Design review of the part built by this model. Coordinates are the model's own, in mm. A direction names the side the tool comes from. Round coordinates to 2 decimals unless told otherwise and drop trailing zeros. Loops run counter-clockwise (first coordinate to the right, second up) from the corner with the lowest first, then second, coordinate; pieces in that order, holes last. Notation, with made-up numbers: (9, -14.75) - (39, -14.75) arc R15 cw to (39, 5.25) - close; hole circle Ø8 at (28.5, -34). An arc over 180 degrees is marked (long way). Return JSON: item names as keys, results as strings. Group by question number.
(1) For faces 4 (the flat face through (10, 158, 20)), 5 (the flat face through (15, 158, 10.3)), list the 3-axis set-ups (+Z, -Z, +X, -X, +Y, -Y) from which the entire face can be reached by the end or side of a thin tool; tool diameter is ignored.
(2) We need section C-C, the plane y = 124.5. Give the number of separate pieces and of enclosed holes in the cut face, and give its area (3 significant figures).
(3) Clearance check with flat-ended pins moving along their axes: pin 1 (0.8 mm diameter, centred on y = 181, z = 17.5, fed in from +X); pin 2 (0.8 mm diameter, centred on y = 106, z = 18.5, fed in from -X); pin 3 (1.1 mm diameter, centred on y = 237.5, z = 4.5, fed in from -X). State where each tip first meets the part, or that it passes through.
(4) Wall thickness on L1, parallel to Z at x = 15, y = 106; L2, parallel to Z at x = 15.5, y = 204.5: over which ranges is each line inside the solid? List them lowest first. Write a range as [from, to].
(5) We need section A-A, the plane x = 0. Write out the cut boundary in (y, z), and give its area (3 significant figures).
(6) The part is to be moulded in two halves that separate along X. For faces 1 (the cylindrical face through (13.94, 157.76, -13.03)), 2 (the flat face through (10, 158, -20)), 3 (the flat face through (-20, 158, 10)), say which applies: pulls with the +X half, pulls with the -X half, needs draft (parallel to the pull), parting line crosses it, or undercut.
(7) We need section B-B, the plane z = 0. Write out the cut boundary in (x, y).
from build123d import *

# Parameters (mm, degrees)
SKETCH16_R     = 3.4
SKETCH16_R_2   = 3
MEMBER_1_DEPTH = 320


with BuildPart() as part:
    # Sketch16 → Member 1 (new body)
    with BuildSketch(Plane(origin=(0, 0, 0), x_dir=(-1, 0, 0), z_dir=(0, 1, 0))):
        with BuildLine():
            Line((-5.1, 20), (-5.1, 19.5))
            Line((-5.1, 19.5), (-4.1, 19.5))
            Line((-4.1, 19.5), (-4.1, 17))
            Line((-4.1, 17), (-6.1, 17))
            Line((-6.1, 17), (-6.1, 18))
            Line((-6.1, 18), (-10.3, 18))
            Line((-10.3, 18), (-10.3, 12))
            Line((-10.3, 12), (-6, 7.7))
            Line((-6, 7.7), (6, 7.7))
            Line((6, 7.7), (10.3, 12))
            Line((10.3, 12), (10.3, 18))
            Line((10.3, 18), (6.1, 18))
            Line((6.1, 18), (6.1, 17))
            Line((6.1, 17), (4.1, 17))
            Line((4.1, 17), (4.1, 19.5))
            Line((4.1, 19.5), (5.1, 19.5))
            Line((5.1, 19.5), (5.1, 20))
            Line((5.1, 20), (15.5, 20))
            ThreePointArc((15.5, 20), (18.681980515, 18.681980515), (20, 15.5))
            Line((20, 15.5), (20, 5.1))
            Line((20, 5.1), (19.5, 5.1))
            Line((19.5, 5.1), (19.5, 4.1))
            Line((19.5, 4.1), (17, 4.1))
            Line((17, 4.1), (17, 6.1))
            Line((17, 6.1), (18, 6.1))
            Line((18, 6.1), (18, 10.3))
            Line((18, 10.3), (12, 10.3))
            Line((12, 10.3), (7.7, 6))
            Line((7.7, 6), (7.7, -6))
            Line((7.7, -6), (12, -10.3))
            Line((12, -10.3), (18, -10.3))
            Line((18, -10.3), (18, -6.1))
            Line((18, -6.1), (17, -6.1))
            Line((17, -6.1), (17, -4.1))
            Line((17, -4.1), (19.5, -4.1))
            Line((19.5, -4.1), (19.5, -5.1))
            Line((19.5, -5.1), (20, -5.1))
            Line((20, -5.1), (20, -15.5))
            ThreePointArc((20, -15.5), (18.681980515, -18.681980515), (15.5, -20))
            Line((15.5, -20), (5.1, -20))
            Line((5.1, -20), (5.1, -19.5))
            Line((5.1, -19.5), (4.1, -19.5))
            Line((4.1, -19.5), (4.1, -17))
            Line((4.1, -17), (6.1, -17))
            Line((6.1, -17), (6.1, -18))
            Line((6.1, -18), (10.3, -18))
            Line((10.3, -18), (10.3, -12))
            Line((10.3, -12), (6, -7.7))
            Line((6, -7.7), (-6, -7.7))
            Line((-6, -7.7), (-10.3, -12))
            Line((-10.3, -12), (-10.3, -18))
            Line((-10.3, -18), (-6.1, -18))
            Line((-6.1, -18), (-6.1, -17))
            Line((-6.1, -17), (-4.1, -17))
            Line((-4.1, -17), (-4.1, -19.5))
            Line((-4.1, -19.5), (-5.1, -19.5))
            Line((-5.1, -19.5), (-5.1, -20))
            Line((-5.1, -20), (-15.5, -20))
            ThreePointArc((-15.5, -20), (-18.681980515, -18.681980515), (-20, -15.5))
            Line((-20, -15.5), (-20, -5.1))
            Line((-20, -5.1), (-19.5, -5.1))
            Line((-19.5, -5.1), (-19.5, -4.1))
            Line((-19.5, -4.1), (-17, -4.1))
            Line((-17, -4.1), (-17, -6.1))
            Line((-17, -6.1), (-18, -6.1))
            Line((-18, -6.1), (-18, -10.3))
            Line((-18, -10.3), (-12, -10.3))
            Line((-12, -10.3), (-7.7, -6))
            Line((-7.7, -6), (-7.7, 6))
            Line((-7.7, 6), (-12, 10.3))
            Line((-12, 10.3), (-18, 10.3))
            Line((-18, 10.3), (-18, 6.1))
            Line((-18, 6.1), (-17, 6.1))
            Line((-17, 6.1), (-17, 4.1))
            Line((-17, 4.1), (-19.5, 4.1))
            Line((-19.5, 4.1), (-19.5, 5.1))
            Line((-19.5, 5.1), (-20, 5.1))
            Line((-20, 5.1), (-20, 15.5))
            ThreePointArc((-20, 15.5), (-18.681980515, 18.681980515), (-15.5, 20))
            Line((-15.5, 20), (-5.1, 20))
        make_face()
        Circle(SKETCH16_R, mode=Mode.SUBTRACT)
        with Locations((-15.556349186, 15.556349186)):
            Circle(SKETCH16_R_2, mode=Mode.SUBTRACT)
        with Locations((15.556349186, 15.556349186)):
            Circle(SKETCH16_R_2, mode=Mode.SUBTRACT)
        with Locations((15.556349186, -15.556349186)):
            Circle(SKETCH16_R_2, mode=Mode.SUBTRACT)
        with Locations((-15.556349186, -15.556349186)):
            Circle(SKETCH16_R_2, mode=Mode.SUBTRACT)
    extrude(amount=MEMBER_1_DEPTH)


solid = part.part
Solutions:
{
 "1": {"face 4": "+Z, +X, -X, +Y, -Y", "face 5": "+Y, -Y"},
 "2": {"separate pieces": "1", "enclosed holes": "5", "area": "605 mm^2"},
 "3": {"pin 1": "x = 19.71", "pin 2": "x = -19.17", "pin 3": "x = -19.5"},
 "4": {"L1": "[-20, -18.5], [-12.61, -10.3], [10.3, 12.61], [18.5, 20]", "L2": "[-20, -18.56], [-12.56, -10.3], [10.3, 12.56], [18.56, 20]"},
 "5": {"outline": "(0, -7.7) - (320, -7.7) - (320, -3.4) - (0, -3.4) - close; (0, 3.4) - (320, 3.4) - (320, 7.7) - (0, 7.7) - close", "area": "2,750 mm^2"},
 "6": {"face 1": "undercut", "face 2": "needs draft", "face 3": "pulls with the -X half"},
 "7": {"outline": "(-7.7, 0) - (-3.4, 0) - (-3.4, 320) - (-7.7, 320) - close; (3.4, 0) - (7.7, 0) - (7.7, 320) - (3.4, 320) - close"}
}
